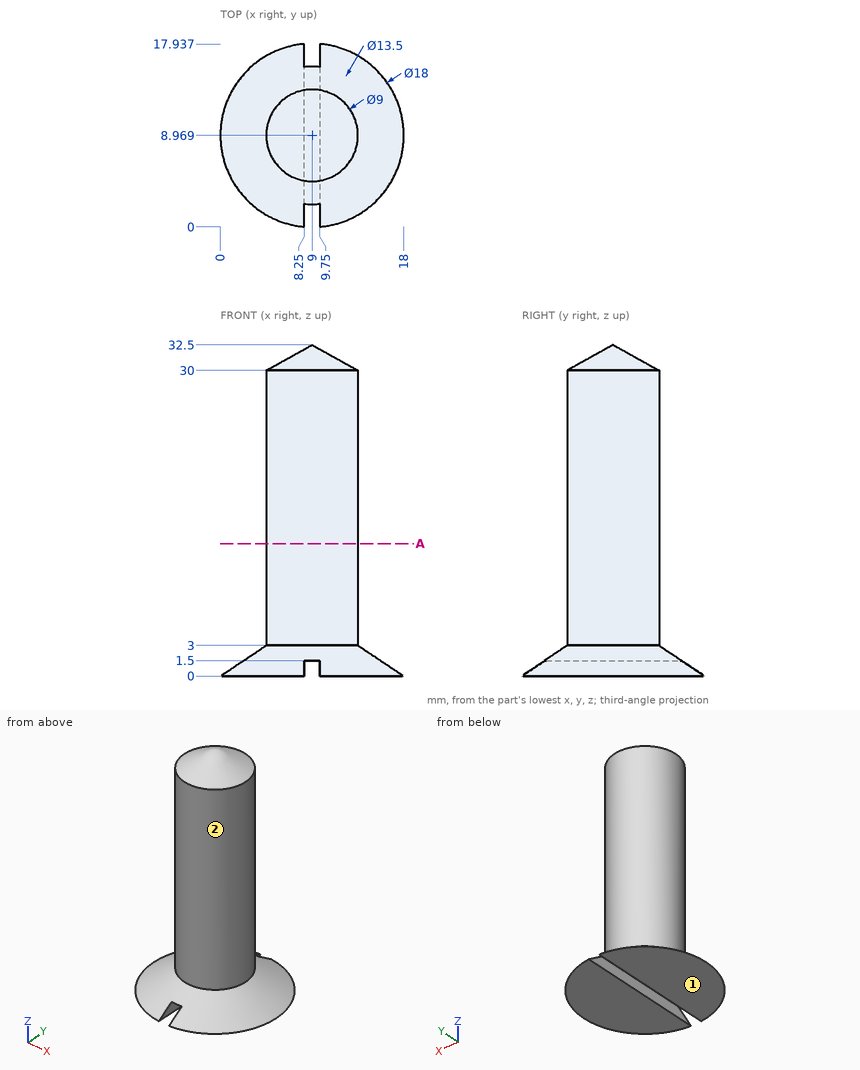
Could you check a few things on this drawing? It's one solid part, dimensions in mm from its lowest x, y, z. A direction names the side the tool comes from. Round coordinates to 2 decimals unless told otherwise and drop trailing zeros. Loops run counter-clockwise (first coordinate to the right, second up) from the corner with the lowest first, then second, coordinate; pieces in that order, holes last. Notation, with made-up numbers: M 80,11 L 92,11 A26 ccw 92,47 Z; hole C 5,-13.75 d7. An arc over 180 degrees is marked long. Write each question's results on one line, items separated by ' | '. Start each with the question number.
(1) Will these pins go through, and if not, where does the flat tip stop? P1, Ø0.5, axis at y = 12, z = 0.5, coming from the +X side (1 decimal); P2, Ø0.8, axis at x = 9, y = 11, coming from the -Z side; P3, Ø2, axis at y = 4, z = 23.5, coming from the +X side.
(2) On a 3-axis mill with a long thin cutter (end or side, diameter ignored), from which of +Z, -Z, +X, -X, +Y, -Y can I reach the whole of each face in a straight line? I mean the marked faces 1 and 2. Say none if no direction works.
(3) I want a section at A-A (z = 13). Please give me the cut outline in (x, y).
(4) If I drill on probe 1 along X at (y, z) = (5.75, 17.5) (1 decimal); probe 2 along X at (y, z) = (10.5, 18.5); probe 3 along Z at (x, y) = (12.5, 10.5), over which ranges is the centre line in solid material (lowest first)? Write a range as from..to.
Solved:
1) P1: stops at x = 17.1 | P2: stops at z = 1.5 | P3: stops at x = 11.12
2) face 1: -Z, +X, -X, +Y, -Y | face 2: +Z
3) outline: C 9,8.97 d9
4) probe 1: x = 5.9..12.1 | probe 2: x = 4.77..13.23 | probe 3: z = 0..30.38
